Input: part model. Units: mm. Frame: model coordinates. A direction names the side the tool comes from. Round coordinates to 2 decimals unless told otherwise and drop trailing zeros. Loops run counter-clockwise (first coordinate to the right, second up) from the corner with the lowest first, then second, coordinate; pieces in that order, holes last. Notation, with made-up numbers: (63.5, 27) - (109.5, 27) arc R10 ccw to (109.5, 44) - close; hole circle Ø1 at (14.25, -26.75). An arc over 180 degrees is marked (long way). One line per question, with ' | ' between items. Start each with the question number.
Item 1: First-contact query: pin 1 (6 mm diameter, centred on x = -3, y = -27.5, fed in from +Z); pin 2 (3.5 mm diameter, centred on x = 47, y = -27.5, fed in from +Z); pin 3 (6 mm diameter, centred on x = 47, y = 22.5, fed in from -Z); pin 4 (9 mm diameter, centred on x = 50, y = 42, fed in from +Z). Flat tips, straight axial feed; report the tip coordinate or a pass-through.
Item 2: Draft query along X for faces 4 (the face through (-1, 47.5, 6)), 5 (the face through (-3.121, -30.247, 8.806)). Return one class per face: pulls with the +X half, pulls with the -X half, needs draft (parallel to the pull), parting line crosses it, or undercut.
Item 3: Section B-B, the plane x = -3. Return loops of the section in (y, z) (3 decimals).
Item 4: Section A-A, the plane z = 1.5. Give the number of separate pieces and of enclosed holes in the cut face, plus the area to 3 significant figures.
Item 5: Set-up query: faces 1 (the face through (-51, -30, 5.7)), 2 (the face through (49.01, 38.35, 2.64)), 3 (the face through (50, -36, 8)). Return all of +Z, -Z, +X, -X, +Y, -Y with unobstructed straight access to the full face (end or side cutting, diameter ignored); none if empty.
Item 6: Section C-C, the plane y = -2.5. Return loops of the section in (x, z), plus the area to 3 significant figures.
Item 7: Material intervals for line 1 along X through (y, z) = (-27.5, 1.85); line 2 along Y through (x, z) = (50, 7); line 3 along X through (y, z) = (22.5, 9), sorted ascending.
```python
from build123d import *

# Parameters (mm, degrees)
SKETCH_1_W               = 150
SKETCH_1_H               = 95
EXTRUDE_1_DEPTH          = 12
HOLE_WIZARD_1_AT_2_COUNT = 2
HOLE_WIZARD_1_AT_2_PITCH = 100
HOLE_WIZARD_1_AT_3_COUNT = 2
HOLE_WIZARD_1_AT_3_PITCH = 83
HOLE_WIZARD_1_AT_4_COUNT = 2
HOLE_WIZARD_1_AT_4_PITCH = 129.957685421
HOLE_WIZARD_2_AT_2_COUNT = 2
HOLE_WIZARD_2_AT_2_PITCH = 50
HOLE_WIZARD_2_AT_3_COUNT = 2
HOLE_WIZARD_2_AT_3_PITCH = 100
HOLE_WIZARD_2_AT_4_COUNT = 2
HOLE_WIZARD_2_AT_4_PITCH = 111.803398875
HOLE_WIZARD_2_AT_5_COUNT = 2
HOLE_WIZARD_2_AT_5_PITCH = 70.710678119
HOLE_WIZARD_2_AT_6_COUNT = 2
HOLE_WIZARD_2_AT_6_PITCH = 50
SKETCH_9_R               = 22.5
CUT_EXTRUDE_1_DEPTH      = 90.583759689


with BuildPart() as part:
    # 草图1 → 凸台-拉伸1 (new body)
    with BuildSketch(Plane.XY):
        Rectangle(SKETCH_1_W, SKETCH_1_H)
    extrude(amount=EXTRUDE_1_DEPTH)

    # 草图6 → 打孔尺寸(%根据)内六角圆柱头螺钉的类型1 (revolve, cut)
    with BuildSketch(Plane(origin=(-50, -41.5, 12), x_dir=(0, -1, 0), z_dir=(1, 0, 0))):
        Polygon((0, 0), (0, 12), (3.3, 12), (3.3, 6.8), (5.5, 6.8), (5.5, 0.9), (6.4, 0), align=None)
    hole_wizard_1 = revolve(axis=Axis((-50, -41.5, 18.35), (0, 0, -1)), mode=Mode.SUBTRACT)

    # 打孔尺寸(%根据)内六角圆柱头螺钉的类型1 at 2: 打孔尺寸(%根据)内六角圆柱头螺钉的类型1 ×2
    with Locations(*[(i * HOLE_WIZARD_1_AT_2_PITCH, 0, 0) for i in range(1, HOLE_WIZARD_1_AT_2_COUNT)]):
        add(hole_wizard_1, mode=Mode.SUBTRACT)

    # 打孔尺寸(%根据)内六角圆柱头螺钉的类型1 at 3: 打孔尺寸(%根据)内六角圆柱头螺钉的类型1 ×2
    with Locations(*[(0, i * HOLE_WIZARD_1_AT_3_PITCH, 0) for i in range(1, HOLE_WIZARD_1_AT_3_COUNT)]):
        add(hole_wizard_1, mode=Mode.SUBTRACT)

    # 打孔尺寸(%根据)内六角圆柱头螺钉的类型1 at 4: 打孔尺寸(%根据)内六角圆柱头螺钉的类型1 ×2
    with Locations(*[Vector(0.7694812328797624, 0.6386694232902033, 0) * (i * HOLE_WIZARD_1_AT_4_PITCH) for i in range(1, HOLE_WIZARD_1_AT_4_COUNT)]):
        add(hole_wizard_1, mode=Mode.SUBTRACT)

    # 草图8 → 打孔尺寸(%根据)内六角圆柱头螺钉的类型2 (revolve, cut)
    with BuildSketch(Plane(origin=(-53, -27.5, 0), x_dir=(0, 1, 0), z_dir=(1, 0, 0))):
        Polygon((0, 0), (0, 12), (2.75, 12), (2.75, 5.7), (5, 5.7), (5, 0.025), (5.025, 0), align=None)
    hole_wizard_2 = revolve(axis=Axis((-53, -27.5, -6.35), (0, 0, 1)), mode=Mode.SUBTRACT)

    # 打孔尺寸(%根据)内六角圆柱头螺钉的类型2 at 2: 打孔尺寸(%根据)内六角圆柱头螺钉的类型2 ×2
    with Locations(*[(i * HOLE_WIZARD_2_AT_2_PITCH, 0, 0) for i in range(1, HOLE_WIZARD_2_AT_2_COUNT)]):
        add(hole_wizard_2, mode=Mode.SUBTRACT)

    # 打孔尺寸(%根据)内六角圆柱头螺钉的类型2 at 3: 打孔尺寸(%根据)内六角圆柱头螺钉的类型2 ×2
    with Locations(*[(i * HOLE_WIZARD_2_AT_3_PITCH, 0, 0) for i in range(1, HOLE_WIZARD_2_AT_3_COUNT)]):
        add(hole_wizard_2, mode=Mode.SUBTRACT)

    # 打孔尺寸(%根据)内六角圆柱头螺钉的类型2 at 4: 打孔尺寸(%根据)内六角圆柱头螺钉的类型2 ×2
    with Locations(*[Vector(0.8944271909999156, 0.4472135954999584, 0) * (i * HOLE_WIZARD_2_AT_4_PITCH) for i in range(1, HOLE_WIZARD_2_AT_4_COUNT)]):
        add(hole_wizard_2, mode=Mode.SUBTRACT)

    # 打孔尺寸(%根据)内六角圆柱头螺钉的类型2 at 5: 打孔尺寸(%根据)内六角圆柱头螺钉的类型2 ×2
    with Locations(*[Vector(0.7071067811865471, 0.7071067811865479, 0) * (i * HOLE_WIZARD_2_AT_5_PITCH) for i in range(1, HOLE_WIZARD_2_AT_5_COUNT)]):
        add(hole_wizard_2, mode=Mode.SUBTRACT)

    # 打孔尺寸(%根据)内六角圆柱头螺钉的类型2 at 6: 打孔尺寸(%根据)内六角圆柱头螺钉的类型2 ×2
    with Locations(*[(0, i * HOLE_WIZARD_2_AT_6_PITCH, 0) for i in range(1, HOLE_WIZARD_2_AT_6_COUNT)]):
        add(hole_wizard_2, mode=Mode.SUBTRACT)

    # 草图9 → 切除-拉伸1 (cut, through all)
    with BuildSketch(Plane(origin=(0, 0, 0), x_dir=(-1, 0, 0), z_dir=(0, 0, -1))):
        with Locations((-22, -2.5)):
            Circle(SKETCH_9_R)
    extrude(amount=-CUT_EXTRUDE_1_DEPTH, mode=Mode.SUBTRACT)


solid = part.part
```
Return value:
1) pin 1: z = 12 | pin 2: through | pin 3: z = 5.7 | pin 4: z = 5.2
2) face 4: needs draft | face 5: undercut
3) outline: (-47.5, 0) - (-32.525, 0) - (-32.5, 0.025) - (-32.5, 5.7) - (-30.25, 5.7) - (-30.25, 12) - (-47.5, 12) - close; (-24.75, 5.7) - (-22.5, 5.7) - (-22.5, 0.025) - (-22.475, 0) - (17.475, 0) - (17.5, 0.025) - (17.5, 5.7) - (19.75, 5.7) - (19.75, 12) - (-24.75, 12) - close; (25.25, 5.7) - (27.5, 5.7) - (27.5, 0.025) - (27.525, 0) - (47.5, 0) - (47.5, 12) - (25.25, 12) - close
4) separate pieces: 1 | enclosed holes: 11 | area: 12,100 mm2
5) face 1: -Z | face 2: +Z, -Z | face 3: +Z
6) outline: (-75, 0) - (-0.5, 0) - (-0.5, 12) - (-75, 12) - close; (44.5, 0) - (75, 0) - (75, 12) - (44.5, 12) - close | area: 1,260 mm2
7) line 1: -75 to -58, -48 to -8, 2 to 42, 52 to 75 | line 2: -47.5 to -47, -36 to 36, 47 to 47.5 | line 3: -75 to -55.75, -50.25 to -5.75, -0.25 to 44.25, 49.75 to 75
